from build123d import *

# Parameters (mm, degrees)
BOSS_EXTRUDE1_DEPTH                                = 20
HOLE_SIZE_BASED_ON_SOCKET_HEAD_CAP_SCR_D           = 3.4
HOLE_SIZE_BASED_ON_SOCKET_HEAD_CAP_SCR_CBORE_D     = 6
HOLE_SIZE_BASED_ON_SOCKET_HEAD_CAP_SCR_CBORE_DEPTH = 10


with BuildPart() as part:
    # Sketch1 → Boss-Extrude1 (new body)
    with BuildSketch(Plane(origin=(0, 0, 0), x_dir=(1, 0, 0), z_dir=(0, 1, 0))):
        with BuildLine():
            Line((-14, 19), (14, 19))
            ThreePointArc((14, 19), (17.535533906, 17.535533906), (19, 14))
            Line((19, 14), (19, -14))
            ThreePointArc((19, -14), (17.535533906, -17.535533906), (14, -19))
            Line((14, -19), (-14, -19))
            ThreePointArc((-14, -19), (-17.535533906, -17.535533906), (-19, -14))
            Line((-19, -14), (-19, 14))
            ThreePointArc((-19, 14), (-17.535533906, 17.535533906), (-14, 19))
        make_face()
    extrude(amount=BOSS_EXTRUDE1_DEPTH)

    # Hole size (%based on) socket head cap screw type 1 (through all)
    with Locations(Plane(origin=(0, 20, 0), x_dir=(1, 0, 0), z_dir=(0, 1, 0))):
        with Locations((-12.5, 12.5), (12.5, 12.5), (12.5, -12.5), (-12.5, -12.5)):
            CounterBoreHole(HOLE_SIZE_BASED_ON_SOCKET_HEAD_CAP_SCR_D / 2, HOLE_SIZE_BASED_ON_SOCKET_HEAD_CAP_SCR_CBORE_D / 2, HOLE_SIZE_BASED_ON_SOCKET_HEAD_CAP_SCR_CBORE_DEPTH)


solid = part.part
Geometry check sheet. Reference: the model listing, model coordinates, mm. A direction names the side the tool comes from. Round coordinates to 2 decimals unless told otherwise and drop trailing zeros. Order: outer loops, then holes, each group sorted by start corner. A loop starts at its lowest first (then second) coordinate and runs counter-clockwise, first axis right, second up. Notation, with made-up numbers: M 88.25,0 L 136.25,0 A11 cw 136.25,15 Z; hole C -10.75,-9 d5. An arc over 180 degrees is marked long. Answer in a Markdown table with one row per item.
(1) Scan lines: probe 1 along Z at (x, y) = (-12.5, 16.5); probe 2 along Z at (x, y) = (12.5, 7.25). Record each from-to range of solid material in increasing order. Write a range as from..to.
Responses:
| item | result |
|---|---|
| probe 1 | z = -19..-15.5, -9.5..9.5, 15.5..19 |
| probe 2 | z = -19..-14.2, -10.8..10.8, 14.2..19 |
(2) Sectioned sample at D-D, the plane y = 9.5. Record the cut outline in (x, z).
Responses:
| item | result |
|---|---|
| outline | M -19,-14 A5 ccw -14,-19 L 14,-19 A5 ccw 19,-14 L 19,14 A5 ccw 14,19 L -14,19 A5 ccw -19,14 Z; hole C -12.5,-12.5 d3.4; hole C -12.5,12.5 d3.4; hole C 12.5,-12.5 d3.4; hole C 12.5,12.5 d3.4 |
(3) Sectioned sample at A-A, the plane y = 17.75. Record the cut outline in (x, z).
Responses:
| item | result |
|---|---|
| outline | M -19,-14 A5 ccw -14,-19 L 14,-19 A5 ccw 19,-14 L 19,14 A5 ccw 14,19 L -14,19 A5 ccw -19,14 Z; hole C -12.5,-12.5 d6; hole C -12.5,12.5 d6; hole C 12.5,-12.5 d6; hole C 12.5,12.5 d6 |
(4) Go/stop test with flat-tipped pins: P1, Ø6.5, axis at x = -13.5, z = -13, coming from the +Y side; P2, Ø5.5, axis at x = 12.5, z = 12.5, coming from the +Y side; P3, Ø2.5, axis at x = -12.5, z = -12.5, coming from the +Y side. Record where each tip stops, or that it passes through.
Responses:
| item | result |
|---|---|
| P1 | stops at y = 20 |
| P2 | stops at y = 10 |
| P3 | passes through |
(5) Draft check along X on faces 1 (the face through (0, 10, -19)), 2 (the face through (17, 10, -18)), 3 (the face through (-11, 10, -11)), 4 (the face through (-14.9, 15.1, 14.3)). Enter one of: released by +X, released by -X, zero draft, split by the parting line, or undercut.
Responses:
| item | result |
|---|---|
| face 1 | zero draft |
| face 2 | released by +X |
| face 3 | undercut |
| face 4 | undercut |
(6) Sectioned sample at C-C, the plane z = -12.5. Record the cut outline in (x, y).
Responses:
| item | result |
|---|---|
| outline | M -19,0 L -14.2,0 L -14.2,10 L -15.5,10 L -15.5,20 L -19,20 Z; M -10.8,0 L 10.8,0 L 10.8,10 L 9.5,10 L 9.5,20 L -9.5,20 L -9.5,10 L -10.8,10 Z; M 14.2,0 L 19,0 L 19,20 L 15.5,20 L 15.5,10 L 14.2,10 Z |
(7) Sectioned sample at B-B, the plane x = -12.5. Record the cut outline in (y, z), and give its area (3 significant figures).
Responses:
| item | result |
|---|---|
| outline | M 0,-19 L 20,-19 L 20,-15.5 L 10,-15.5 L 10,-14.2 L 0,-14.2 Z; M 0,-10.8 L 10,-10.8 L 10,-9.5 L 20,-9.5 L 20,9.5 L 10,9.5 L 10,10.8 L 0,10.8 Z; M 0,14.2 L 10,14.2 L 10,15.5 L 20,15.5 L 20,19 L 0,19 Z |
| area | 572 mm² |
(8) Tool access check on faces 5 (the face through (19, 10, 0)), 6 (the face through (14, 10, 14)). Record the directions out of +Z, -Z, +X, -X, +Y, -Y that give a thin tool (end or side, any length) a straight path to the whole face; none if there is none.
Responses:
| item | result |
|---|---|
| face 5 | +Z, -Z, +X, +Y, -Y |
| face 6 | +Y |
